Can you work these out from the model? Positions are in its coordinate system, mm. Round coordinates to 2 decimals unless told otherwise and drop trailing zeros. Order: outer loops, then holes, each group sorted by start corner. A loop starts at its lowest first (then second) coordinate and runs counter-clockwise, first axis right, second up. Notation, with made-up numbers: (17.5, 52.5) -> (70.5, 52.5) arc R23 ccw to (70.5, 75.5) -> close; hole circle Ø10 at (51.25, -22.75). An arc over 180 degrees is marked (long way). One line per item, written item: value.
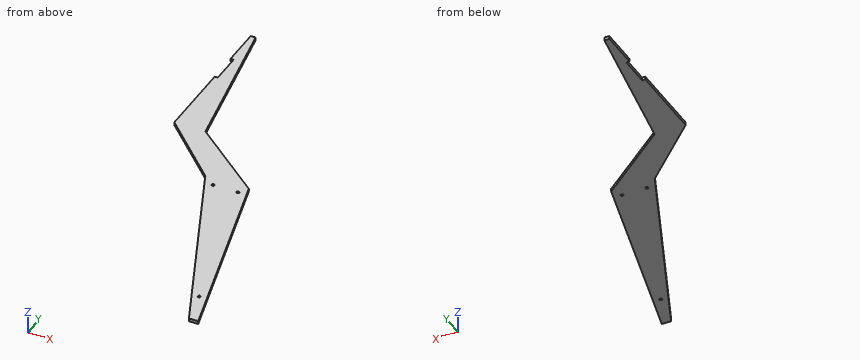
```python
from build123d import *

# Parameters (mm, degrees)
EXTRUDE_1_DEPTH     = 2.5
SKETCH_2_R          = 2.2
CUT_EXTRUDE_1_DEPTH = 10
SKETCH_3_R          = 2.2
CUT_EXTRUDE_2_DEPTH = 10


with BuildPart() as part:
    # 草图1 → 凸台-拉伸1 (new, symmetric)
    with BuildSketch(Plane.XY):
        Polygon((0, 0), (8, 0), (50, -240), (170, -338), (255, -663), (240, -663), (100, -338), (0, -240), (0, -113), (5, -113), (5, -63), (0, -63), align=None)
    extrude(amount=EXTRUDE_1_DEPTH, both=True)

    # 草图2 → 切除-拉伸1 (cut)
    with BuildSketch(Plane.XY.offset(2.5)):
        with Locations((120.192307692, -353)):
            Circle(SKETCH_2_R)
        with Locations((160.192307692, -353)):
            Circle(SKETCH_2_R)
    extrude(amount=-CUT_EXTRUDE_1_DEPTH, mode=Mode.SUBTRACT)

    # 草图3 → 切除-拉伸2 (cut)
    with BuildSketch(Plane.XY.offset(2.5)):
        with Locations((228.461538462, -608)):
            Circle(SKETCH_3_R)
    extrude(amount=-CUT_EXTRUDE_2_DEPTH, mode=Mode.SUBTRACT)


solid = part.part
```
Q1. I want a section at C-C on y = -211. List the corners of the cut face in (x, z) for me (3 decimals), plus the area to 3 significant figures.
Answers below:
outline: (0, -2.5) -> (44.925, -2.5) -> (44.925, 2.5) -> (0, 2.5) -> close
area: 225 mm^2
Q2. I want a section at A-A on z = -0.45. List the corners of the cut face in (x, y) for me.
Answers below:
outline: (0, -240) -> (100, -338) -> (240, -663) -> (255, -663) -> (170, -338) -> (50, -240) -> (8, 0) -> (0, 0) -> (0, -63) -> (5, -63) -> (5, -113) -> (0, -113) -> close; hole circle Ø4.4 at (120.19, -353); hole circle Ø4.4 at (160.19, -353); hole circle Ø4.4 at (228.46, -608)
Q3. I want a section at B-B on x = 78. List the corners of the cut face in (y, z) for me.
Answers below:
outline: (-316.44, -2.5) -> (-262.87, -2.5) -> (-262.87, 2.5) -> (-316.44, 2.5) -> close
Q4. Will these pins go through, and if not, where does the flat tip stop? pin 1 Ø1.5 at (x, z) = (2, -0.5) entering from -Y (3 decimals); pin 2 Ø1 at (x, z) = (89.5, -0.5) entering from -Y; pin 3 Ø1.5 at (x, z) = (90.5, -0.5) entering from -Y (3 decimals).
Answers below:
pin 1: y = -242.695
pin 2: y = -328.2
pin 3: y = -329.425
Q5. Please list where these lines run through material, in increasing order: line 1 along X through (y, z) = (-353, 1.05); line 2 along X through (y, z) = (-609, -1.85); line 3 along X through (y, z) = (-608, -0.65).
Answers below:
line 1: 106.46 to 117.99, 122.39 to 157.99, 162.39 to 173.92
line 2: 216.74 to 226.5, 230.42 to 240.88
line 3: 216.31 to 226.26, 230.66 to 240.62
